For this review, take the finished solid that the model builds, in its own axes (mm). Face numbers are marked on the shaded views. A direction names the side the tool comes from. Give positions to 0.01 mm unless a question says otherwise; leave off trailing zeros. Loops run counter-clockwise (first coordinate to the right, second up) from the corner with the lowest first, then second, coordinate; pieces in that order, holes last. Notation, with made-up numbers: (-6.5, -26) - (40.5, -26) arc R22 ccw to (40.5, -3) - close; hole circle Ø10 at (65.5, 30). An arc over 180 degrees is marked (long way). Put each result on its own line as item: value.
from build123d import *

# Parameters (mm, degrees)
SKETCH1_R           = 45
SKETCH1_R_2         = 27.5
BOSS_EXTRUDE1_DEPTH = 28
CUT_EXTRUDE1_START  = -20
SKETCH2_R           = 45
SKETCH2_R_2         = 35
CUT_EXTRUDE1_DEPTH  = 20
CHAMFER1_SIZE       = 2


with BuildPart() as part:
    # Sketch1 → Boss-Extrude1 (new body)
    with BuildSketch(Plane.XY):
        Circle(SKETCH1_R)
        Circle(SKETCH1_R_2, mode=Mode.SUBTRACT)
    extrude(amount=BOSS_EXTRUDE1_DEPTH)

    # Sketch2 → Cut-Extrude1 (cut)
    with BuildSketch(Plane.XY.offset(28).offset(CUT_EXTRUDE1_START)):
        Circle(SKETCH2_R)
        Circle(SKETCH2_R_2, mode=Mode.SUBTRACT)
    extrude(amount=CUT_EXTRUDE1_DEPTH, mode=Mode.SUBTRACT)

    # Chamfer1
    chamfer1_edges = [part.edges().sort_by_distance(p)[0] for p in [
        (-27.5, 0, 28),
    ]]
    chamfer(chamfer1_edges, length=CHAMFER1_SIZE)


solid = part.part
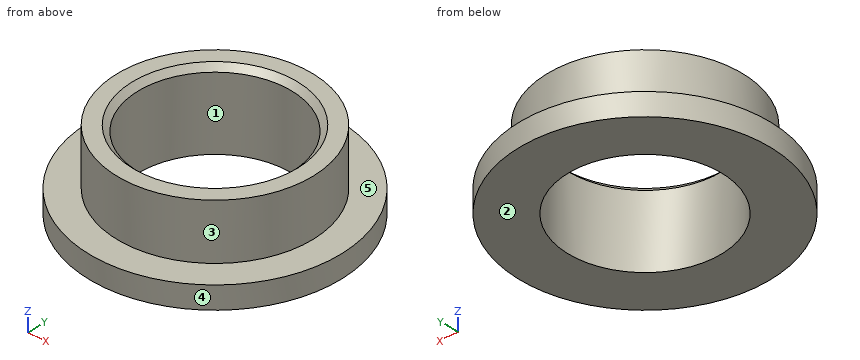
1) Insertion check: pin 1 Ø3 at (x, z) = (25.5, 5) entering from +Y; pin 2 Ø6 at (y, z) = (-21.5, 18.5) entering from +X; pin 3 Ø6 at (y, z) = (-23, 17.5) entering from +X. Each pin has a flat end and moves straight along its axis. Give the tip position at first contact, or say it passes through.
Geometry check:
pin 1: stops at y = 38.07
pin 2: stops at x = 29.71
pin 3: stops at x = 28.72
2) Take a section at A-A on x = 0. State the section outline as (y, z) points.
Geometry check:
outline: (-45, 0) - (-27.5, 0) - (-27.5, 26) - (-29.5, 28) - (-35, 28) - (-35, 8) - (-45, 8) - close; (27.5, 0) - (45, 0) - (45, 8) - (35, 8) - (35, 28) - (29.5, 28) - (27.5, 26) - close
3) Draft analysis for pull direction Y (two halves, no side actions). For the marked faces 1, 2 and 3, state which applies: pulls with the +Y half, pulls with the -Y half, needs draft (parallel to the pull), parting line crosses it, or undercut.
Geometry check:
face 1: undercut
face 2: needs draft
face 3: parting line crosses it
4) Take a section at B-B on y = 31.5. State the section outline as (x, z) points, and give its area (3 significant figures).
Geometry check:
outline: (-32.14, 0) - (32.14, 0) - (32.14, 8) - (15.26, 8) - (15.26, 28) - (-15.26, 28) - (-15.26, 8) - (-32.14, 8) - close
area: 1,120 mm²
5) For the marked faces 4 and 5, list the 3-axis set-ups (+Z, -Z, +X, -X, +Y, -Y) from which the entire face can be reached by the end or side of a thin tool; tool diameter is ignored.
Geometry check:
face 4: +Z, -Z
face 5: +Z
6) Take a section at D-D on x = -38.5. State the section outline as (y, z) points, and give its area (3 significant figures).
Geometry check:
outline: (-23.3, 0) - (23.3, 0) - (23.3, 8) - (-23.3, 8) - close
area: 373 mm²
7) Wall thickness on line 1 (Y direction, x = 0, z = 16.25); line 2 (Y direction, x = 0, z = 7.25); line 3 (Z direction, x = -40, y = 17): over which ranges is each line inside the solid? List them lowest first.
Geometry check:
line 1: y = -35 to -27.5, 27.5 to 35
line 2: y = -45 to -27.5, 27.5 to 45
line 3: z = 0 to 8
8) Take a section at C-C on z = 13. State the section outline as (x, y) points, and give its area (3 significant figures).
Geometry check:
outline: circle Ø70 at (0, 0); hole circle Ø55 at (0, 0)
area: 1,470 mm²
